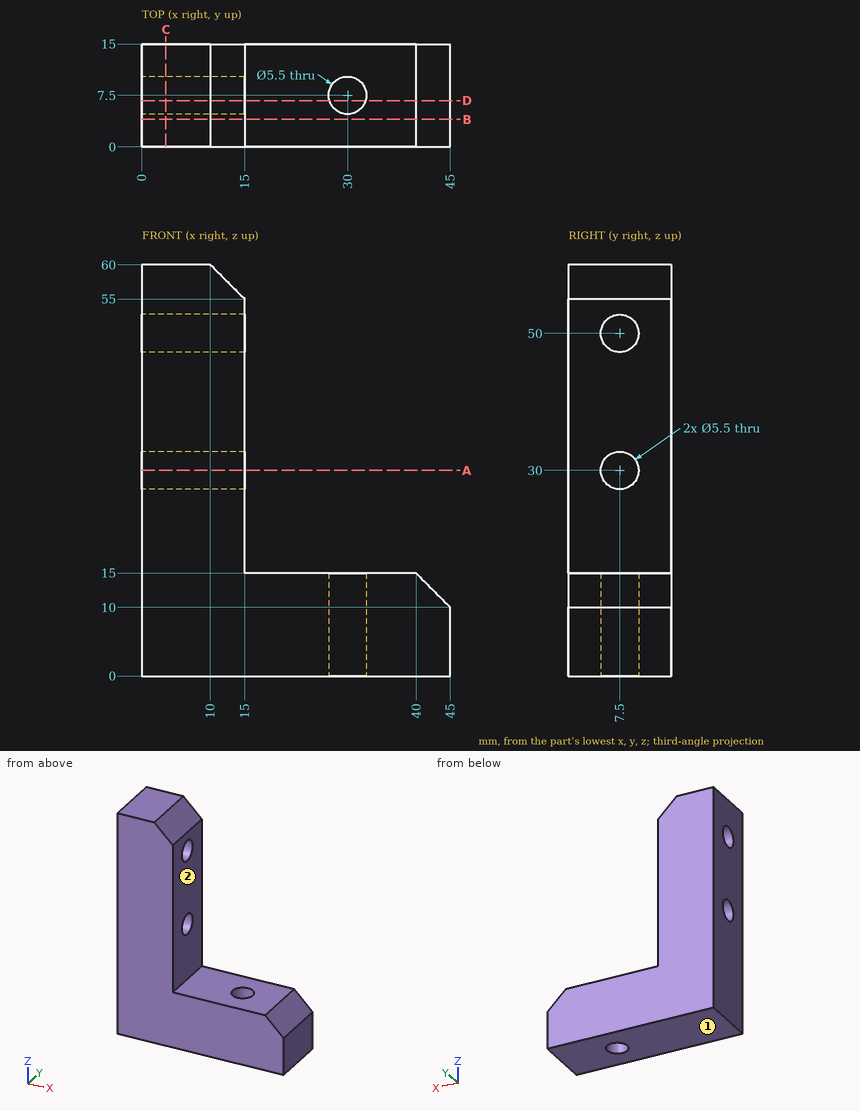
Drawing for the job (mm, zero at the part's lowest x, y, z). A direction names the side the tool comes from. Give positions to 0.01 mm unless a question says otherwise; leave off trailing zeros. Loops run counter-clockwise (first coordinate to the right, second up) from the corner with the lowest first, then second, coordinate; pieces in that order, holes last. Notation, with made-up numbers: M -14.5,56 L 33.5,56 A19 ccw 33.5,83 Z; hole C 17,18.25 d6. An arc over 180 degrees is marked long. One line per question, with ' | ' between items. Start each with the question number.
1. Saw through at D-D on y = 6.75. Give the cut face in (x, z).
2. Saw through at A-A on z = 30. Give the cut face in (x, y).
3. Probe L1, parallel to Y at x = 3, z = 30; L2, parallel to Z at x = 8, y = 10; L3, parallel to X at y = 5.5, z = 53.5. List the from-to ranges inside material, lowest first. Write a range as from..to.
4. Saw through at C-C on x = 3.5. Give the cut face in (y, z).
5. Saw through at B-B on y = 4. Give the cut face in (x, z).
6. Flat gauge pins, fed straight in: pin 1 (6 mm diameter, centred on x = 9.5, y = 6, fed in from -Z); pin 2 (3.5 mm diameter, centred on y = 7.5, z = 30, fed in from +X); pin 3 (2 mm diameter, centred on x = 21.5, y = 7, fed in from +Z); pin 4 (2 mm diameter, centred on y = 11, z = 29, fed in from +X). Where does each tip first touch, or does it go through?
7. 3-axis set-ups, long thin cutter, end or side, ignore diameter. For the marked faces 1 and 2: which of +Z, -Z, +X, -X, +Y, -Y reach the whole face in a straight line?
Result sheet:
1) outline: M 0,0 L 27.35,0 L 27.35,15 L 15,15 L 15,27.35 L 0,27.35 Z; M 0,32.65 L 15,32.65 L 15,47.35 L 0,47.35 Z; M 0,52.65 L 15,52.65 L 15,55 L 10,60 L 0,60 Z; M 32.65,0 L 45,0 L 45,10 L 40,15 L 32.65,15 Z
2) outline: M 0,0 L 15,0 L 15,4.75 L 0,4.75 Z; M 0,10.25 L 15,10.25 L 15,15 L 0,15 Z
3) L1: y = 0..4.75, 10.25..15 | L2: z = 0..28.85, 31.15..48.85, 51.15..60 | L3: x = 0..15
4) outline: M 0,0 L 15,0 L 15,60 L 0,60 Z; hole C 7.5,30 d5.5; hole C 7.5,50 d5.5
5) outline: M 0,0 L 45,0 L 45,10 L 40,15 L 15,15 L 15,55 L 10,60 L 0,60 Z
6) pin 1: stops at z = 0 | pin 2: passes through | pin 3: stops at z = 15 | pin 4: stops at x = 15
7) face 1: -Z, +X, -X, +Y, -Y | face 2: +Z, +X, +Y, -Y
